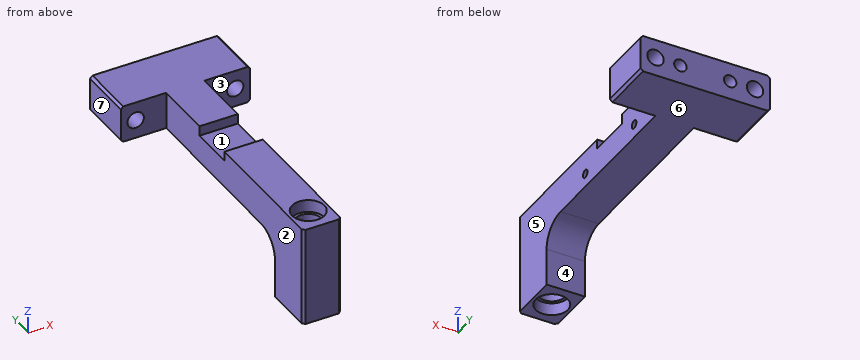
from build123d import *

# Parameters (mm, degrees)
SKETCH1_W                     = 52
SKETCH1_H                     = 120
BOSS_EXTRUDE1_DEPTH           = 7.5
SKETCH8_W                     = 18.3
SKETCH8_H                     = 98
CUT_EXTRUDE4_DEPTH            = 68.089492471
F_6_6_6_6_DIAMETER_HOLE1_D    = 6.6
CHAMFER1_SIZE                 = 1
BLIND_PIN_HOLE1_SIZE_MM_D     = 5
BLIND_PIN_HOLE1_SIZE_MM_DEPTH = 11
BLIND_PIN_HOLE1_SIZE_MM_TIP   = 1.502151548
BOSS_EXTRUDE2_DEPTH           = 25
FILLET1_R                     = 10
SKETCH14_R                    = 5.25
CUT_EXTRUDE5_DEPTH            = 77.655071587
SKETCH15_R                    = 6.5
CUT_EXTRUDE6_DEPTH            = 5
CUT_EXTRUDE7_START            = -5
SKETCH16_R                    = 6.5
CUT_EXTRUDE7_DEPTH            = 5
SKETCH17_W                    = 4
SKETCH17_H                    = 18
CUT_EXTRUDE8_DEPTH            = 77.104796169
M4_TAPPED_HOLE1_D             = 3.3
M4_TAPPED_HOLE1_DEPTH         = 10.1
M4_TAPPED_HOLE1_TIP           = 0.991420021


with BuildPart() as part:
    # Sketch1 → Boss-Extrude1 (new, symmetric)
    with BuildSketch(Plane.XY):
        Rectangle(SKETCH1_W, SKETCH1_H)
    extrude(amount=BOSS_EXTRUDE1_DEPTH, both=True)

    # Sketch8 → Cut-Extrude4 (cut, through all)
    with BuildSketch(Plane.XY.offset(7.5)):
        with Locations((-16.85, -11)):
            Rectangle(SKETCH8_W, SKETCH8_H)
    cut_extrude4 = extrude(amount=-CUT_EXTRUDE4_DEPTH, mode=Mode.SUBTRACT)

    # Mirror1: Cut-Extrude4 across plane
    add(cut_extrude4.mirror(Plane(origin=(0, 0, 0), x_dir=(0, 0, 1), z_dir=(1, 0, 0))), mode=Mode.SUBTRACT)

    # Ø6.6 (6.6) Diameter Hole1 (through all)
    with Locations(Plane(origin=(0, 60, 0), x_dir=(1, 0, 0), z_dir=(0, 1, 0))):
        with Locations((-20, 0), (20, 0)):
            Hole(F_6_6_6_6_DIAMETER_HOLE1_D / 2)

    # Chamfer1
    chamfer1_edges = [part.edges().sort_by_distance(p)[0] for p in [
        (-26, 49, 7.5),
        (-7.7, -60, 0),
        (26, 49, -7.5),
        (26, 49, 7.5),
        (7.7, -60, 0),
        (-26, 49, -7.5),
    ]]
    chamfer(chamfer1_edges, length=CHAMFER1_SIZE)

    # Blind Pin Hole1 size mm
    with Locations(Plane(origin=(0, 60, 0), x_dir=(1, 0, 0), z_dir=(0, 1, 0))):
        with Locations((-10, 0), (10, 0)):
            Hole(BLIND_PIN_HOLE1_SIZE_MM_D / 2, depth=BLIND_PIN_HOLE1_SIZE_MM_DEPTH)
            with Locations((0, 0, -(BLIND_PIN_HOLE1_SIZE_MM_DEPTH + BLIND_PIN_HOLE1_SIZE_MM_TIP / 2))):  # 118° drill point
                Cone(0, BLIND_PIN_HOLE1_SIZE_MM_D / 2, BLIND_PIN_HOLE1_SIZE_MM_TIP, mode=Mode.SUBTRACT)

    # Sketch13 → Boss-Extrude2 (add)
    with BuildSketch(Plane(origin=(0, 0, -7.5), x_dir=(-1, 0, 0), z_dir=(0, 0, -1))):
        Polygon((-7.7, -40), (7.7, -40), (7.7, -59), (6.7, -60), (-6.7, -60), (-7.7, -59), align=None)
    extrude(amount=BOSS_EXTRUDE2_DEPTH)

    # Fillet1
    fillet1_edges = [part.edges().sort_by_distance(p)[0] for p in [
        (0, -40, -7.5),
    ]]
    fillet(fillet1_edges, radius=FILLET1_R)

    # Sketch14 → Cut-Extrude5 (cut, through all)
    with BuildSketch(Plane.XY.offset(7.5)):
        with Locations((0, -50)):
            Circle(SKETCH14_R)
    extrude(amount=-CUT_EXTRUDE5_DEPTH, mode=Mode.SUBTRACT)

    # Sketch15 → Cut-Extrude6 (cut)
    with BuildSketch(Plane.XY.offset(7.5)):
        with Locations((0, -50)):
            Circle(SKETCH15_R)
    extrude(amount=-CUT_EXTRUDE6_DEPTH, mode=Mode.SUBTRACT)

    # Sketch16 → Cut-Extrude7 (cut)
    with BuildSketch(Plane(origin=(0, 0, -32.5), x_dir=(-1, 0, 0), z_dir=(0, 0, -1)).offset(CUT_EXTRUDE7_START)):
        with Locations(Location((0, -50, 0), (0, 0, 180))):
            Circle(SKETCH16_R)
    extrude(amount=CUT_EXTRUDE7_DEPTH, mode=Mode.SUBTRACT)

    # Sketch17 → Cut-Extrude8 (cut, through all)
    with BuildSketch(Plane(origin=(7.7, 0, 0), x_dir=(0, 0, -1), z_dir=(1, 0, 0))):
        with Locations((-5.5, 5.2)):
            Rectangle(SKETCH17_W, SKETCH17_H)
    extrude(amount=-CUT_EXTRUDE8_DEPTH, mode=Mode.SUBTRACT)

    # M4 Tapped Hole1
    with Locations(Plane(origin=(7.7, 0, 0), x_dir=(0, 0, -1), z_dir=(1, 0, 0))):
        with Locations((2, 22.7), (2, -12.3)):
            Hole(M4_TAPPED_HOLE1_D / 2, depth=M4_TAPPED_HOLE1_DEPTH)
            with Locations((0, 0, -(M4_TAPPED_HOLE1_DEPTH + M4_TAPPED_HOLE1_TIP / 2))):  # 118° drill point
                Cone(0, M4_TAPPED_HOLE1_D / 2, M4_TAPPED_HOLE1_TIP, mode=Mode.SUBTRACT)


solid = part.part
Read the model definition and answer for the solid it produces. Units are mm, in the model's axes. Face numbers are marked on the shaded views. A direction names the side the tool comes from. Coordinates: 2 decimals unless noted, no trailing zeros. Write each loop counter-clockwise with the first axis right and the second up, starting at its lowest first coordinate (ties: lowest second). Pieces come first, ordered by that corner, then holes. Notation, with made-up numbers: (-1, -3.5) - (16, -3.5) arc R26 ccw to (16, 31.5) - close; hole circle Ø7 at (36.25, 40.25). An arc over 180 degrees is marked (long way). One line per question, with ' | ' between items.
Q1. Each of these flat-tipped pins is pushed along its axis until it touches: P1, Ø9.5, axis at x = 0, y = -50, coming from the -Z side; P2, Ø2.5, axis at y = -12.3, z = -2, coming from the +X side; P3, Ø10.5, axis at x = -2.5, y = -50.5, coming from the +Z side; P4, Ø20, axis at y = -12, z = -7, coming from the -X side. Where does it stop, or does it pass through?
Result set:
P1: through | P2: x = -2.64 | P3: z = 7.5 | P4: x = -7.7
Q2. Find section A-A, the plane y = -50. Write down the section's boundary in (x, z), plus the area to 3 significant figures.
Result set:
outline: (-7.7, -32.5) - (-6.5, -32.5) - (-6.5, -27.5) - (-5.25, -27.5) - (-5.25, 2.5) - (-6.5, 2.5) - (-6.5, 7.5) - (-7.7, 7.5) - close; (5.25, -27.5) - (6.5, -27.5) - (6.5, -32.5) - (7.7, -32.5) - (7.7, 7.5) - (6.5, 7.5) - (6.5, 2.5) - (5.25, 2.5) - close | area: 171 mm^2
Q3. For the marked faces 1, 2, 3 and 4, determine the directions among +Z, -Z, +X, -X, +Y, -Y from which every point of the face is accessible in a straight line to the end or side of a thin tool.
Result set:
face 1: +Z, +X, -X | face 2: +Z, -Z, -X, -Y | face 3: +Z, -Z, +X, -Y | face 4: -Z, +X, -X, +Y
Q4. Find section B-B, the plane x = -20. Write down the section's boundary in (y, z).
Result set:
outline: (38, -7.5) - (60, -7.5) - (60, -3.3) - (38, -3.3) - close; (38, 3.3) - (60, 3.3) - (60, 7.5) - (38, 7.5) - close
Q5. Consider L1, parallel to Y at x = 0, z = -30; L2, parallel to Z at x = -3, y = -0.5; L3, parallel to Y at x = -21, z = 5. Determine where each line is inside the solid, lowest interval first. Write a range as [from, to].
Result set:
L1: [-60, -56.5], [-43.5, -40] | L2: [-7.5, 3.5] | L3: [38, 60]
Q6. Find section D-D, the plane z = -5. Write down the section's boundary in (x, y).
Result set:
outline: (-26, 38) - (-7.7, 38) - (-7.7, -59) - (-6.7, -60) - (6.7, -60) - (7.7, -59) - (7.7, 38) - (26, 38) - (26, 60) - (-26, 60) - close; hole circle Ø10.5 at (0, -50)
Q7. Determine the mould class of the marked faces 5, 6 and 7 for opening direction X: +X half, -X half, draft (parallel to the pull), parting line (faces both ways), or undercut.
Result set:
face 5: +X half | face 6: draft | face 7: -X half
Q8. Find section C-C, the plane y = 51. Write down the section's boundary in (x, z), plus the area to 3 significant figures.
Result set:
outline: (-26, -6.5) - (-25, -7.5) - (25, -7.5) - (26, -6.5) - (26, 6.5) - (25, 7.5) - (-25, 7.5) - (-26, 6.5) - close; hole circle Ø6.6 at (-20, 0); hole circle Ø5 at (-10, 0); hole circle Ø5 at (10, 0); hole circle Ø6.6 at (20, 0) | area: 670 mm^2
